Could you check a few things on this drawing? It's one solid part, dimensions in mm from its lowest x, y, z. Give positions to 0.01 mm unless a question says otherwise; leave off trailing zeros. Loops run counter-clockwise (first coordinate to the right, second up) from the corner with the lowest first, then second, coordinate; pieces in that order, holes last. Notation, with made-up numbers: (79.25, 67.25) - (116.25, 67.25) arc R25 cw to (116.25, 81.25) - close; hole circle Ø5 at (-19.75, 21.25). An arc over 180 degrees is marked (long way). Return JSON: item names as keys, results as strings. Group by question number.
(1) For P1, Ø8, axis at y = 36.5, z = 45, coming from the -X side; P2, Ø3, axis at x = 10, y = 15.5, coming from the +Z side; P3, Ø9, axis at y = 8, z = 12, coming from the +X side; P4, Ø10, axis at x = 3, y = 56, coming from the -Z side, each with a flat end and sliding along its axis, tell me the tip position at first contact or that it passes through.
(2) If we section it at C-C (x = 12): Please give me the cut outline in (y, z), then the cut area to 3 significant figures.
(3) If we section it at D-D (y = 40): Please give me the cut outline in (x, z), then the cut area to 3 significant figures.
(4) I need wall thicknesses on probe 1 along Z at (x, y) = (12.5, 72); probe 2 along Y at (x, z) = (8.5, 53.5); probe 3 along Y at (x, z) = (3.5, 11). Which ranges of each line are inside material? Lowest first, please. Write a range as [from, to].
(5) If we section it at A-A (z = 12): Please give me the cut outline in (x, y).
(6) If we mould it in two halves opening along Y, with no side actions, what happens to the marked faces 1, 2 and 3? For each: released by +Y, released by -Y, zero draft, split by the parting line, or undercut.
(7) If we section it at B-B (y = 72): Please give me the cut outline in (x, z), then the cut area to 3 significant figures.
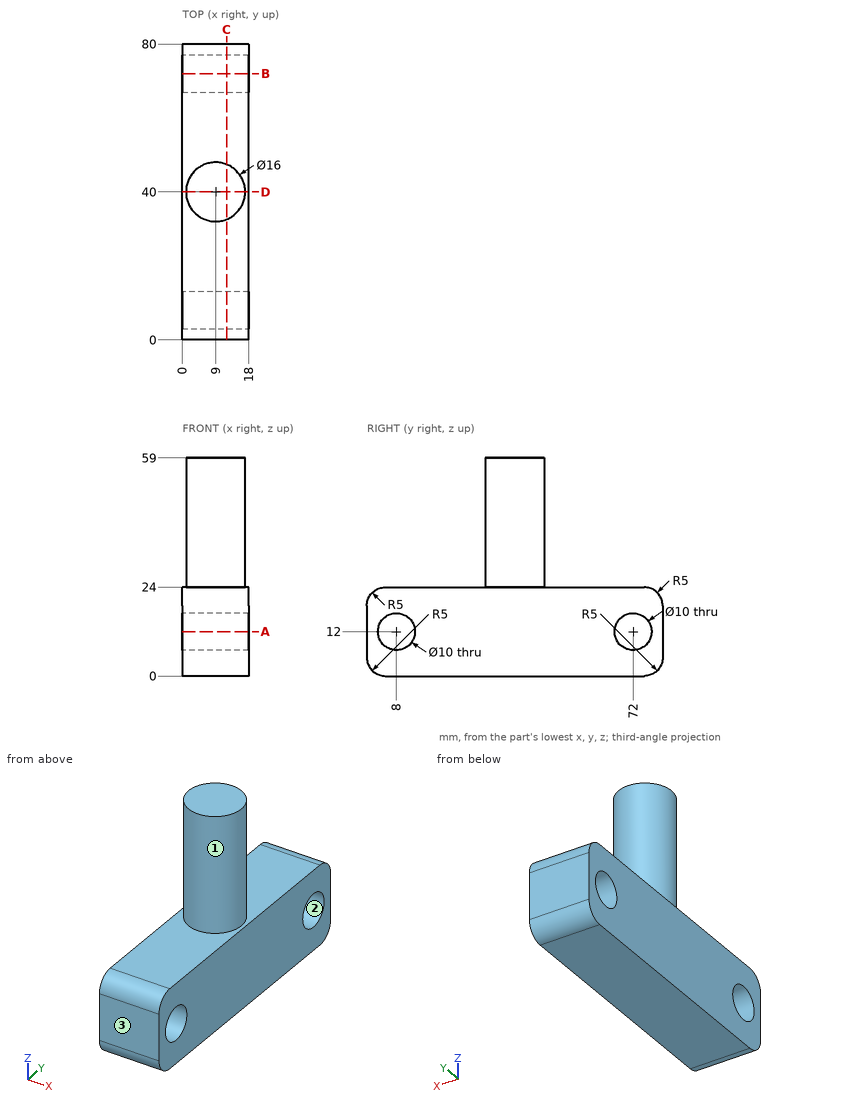
Values:
{
 "1": {"P1": "x = 1", "P2": "z = 24", "P3": "through", "P4": "z = 0"},
 "2": {"outline": "(0, 5) arc R5 ccw to (5, 0) - (75, 0) arc R5 ccw to (80, 5) - (80, 19) arc R5 ccw to (75, 24) - (47.42, 24) - (47.42, 59) - (32.58, 59) - (32.58, 24) - (5, 24) arc R5 ccw to (0, 19) - close; hole circle Ø10 at (8, 12); hole circle Ø10 at (72, 12)", "area": "2,260 mm2"},
 "3": {"outline": "(0, 0) - (18, 0) - (18, 24) - (17, 24) - (17, 59) - (1, 59) - (1, 24) - (0, 24) - close", "area": "992 mm2"},
 "4": {"probe 1": "[0, 7], [17, 24]", "probe 2": "[32.02, 47.98]", "probe 3": "[0, 3.1], [12.9, 67.1], [76.9, 80]"},
 "5": {"outline": "(0, 0) - (18, 0) - (18, 3) - (0, 3) - close; (0, 13) - (18, 13) - (18, 67) - (0, 67) - close; (0, 77) - (18, 77) - (18, 80) - (0, 80) - close"},
 "6": {"face 1": "split by the parting line", "face 2": "undercut", "face 3": "released by -Y"},
 "7": {"outline": "(0, 0) - (18, 0) - (18, 7) - (0, 7) - close; (0, 17) - (18, 17) - (18, 24) - (0, 24) - close", "area": "252 mm2"}
}
